Read the model definition and answer for the solid it produces. Units are mm, in the model's axes. A direction names the side the tool comes from. Coordinates: 2 decimals unless noted, no trailing zeros. Write each loop counter-clockwise with the first axis right and the second up, starting at its lowest first coordinate (ties: lowest second). Pieces come first, ordered by that corner, then holes.
from build123d import *

# Parameters (mm, degrees)
BASE_PLATE_PROFILE_R      = 7.492267371
BASE_PLATE_20MM_DEPTH     = 20
HINGE_KNUCKLE_PROFILE_R   = 10.5
HINGE_KNUCKLE_145MM_DEPTH = 72.5


with BuildPart() as part:
    # Base Plate Profile → Base Plate 20mm (new body)
    with BuildSketch(Plane.XY):
        with BuildLine():
            Line((-72.5, 28.064546487), (72.5, 28.064546487))
            Line((72.5, 28.064546487), (72.5, -16.935453513))
            ThreePointArc((72.5, -16.935453513), (69.894587599, -26.538447706), (62.792895003, -33.507782934))
            Line((62.792895003, -33.507782934), (9.292895003, -63.507782934))
            ThreePointArc((9.292895003, -63.507782934), (0, -65.935453513), (-9.292895003, -63.507782934))
            Line((-9.292895003, -63.507782934), (-62.792895003, -33.507782934))
            ThreePointArc((-62.792895003, -33.507782934), (-69.894587599, -26.538447706), (-72.5, -16.935453513))
            Line((-72.5, -16.935453513), (-72.5, 28.064546487))
        make_face()
        with Locations((0, -46.935453513)):
            Circle(BASE_PLATE_PROFILE_R, mode=Mode.SUBTRACT)
        with Locations((53.5, -16.935453513)):
            Circle(BASE_PLATE_PROFILE_R, mode=Mode.SUBTRACT)
        with Locations((-53.5, -16.935453513)):
            Circle(BASE_PLATE_PROFILE_R, mode=Mode.SUBTRACT)
    extrude(amount=BASE_PLATE_20MM_DEPTH)

    # Hinge Knuckle Profile → Hinge Knuckle 145mm (add, symmetric)
    with BuildSketch(Plane(origin=(0, 0, 0), x_dir=(0, 0, -1), z_dir=(1, 0, 0))):
        with BuildLine():
            Line((29, 61.064546487), (29, 28.064546487))
            Line((29, 28.064546487), (-13, 28.064546487))
            Line((-13, 28.064546487), (-13, 61.064546487))
            ThreePointArc((-13, 61.064546487), (8, 82.064546487), (29, 61.064546487))
        make_face()
        with Locations((8, 61.064546487)):
            Circle(HINGE_KNUCKLE_PROFILE_R, mode=Mode.SUBTRACT)
    extrude(amount=HINGE_KNUCKLE_145MM_DEPTH, both=True)


solid = part.part
Item 1: Determine the mould class of faces 1 (the cylindrical face through (-0.975, -39.507, 9.86)), 2 (the flat face through (72.5, 33, 1)), 3 (the cylindrical face through (-1.015, 54.675, 0.332)) for opening direction X: +X half, -X half, draft (parallel to the pull), parting line (faces both ways), or undercut.
Item 2: The part is cut by section A-A (x = 0). Give the vertices of the cut face in (y, z).
Item 3: The part is cut by section B-B (z = -8). Give the vertices of the cut face in (x, y), and give its area (4 significant figures).
Item 4: Given pin 1 (19.5 mm diameter, centred on x = 0, y = -46.94, fed in from -Z); pin 2 (4 mm diameter, centred on x = 22, z = -16, fed in from +Y); pin 3 (12 mm diameter, centred on x = 35.5, z = -6, fed in from +Y); pin 4 (24 mm diameter, centred on x = -53.5, y = -16.94, fed in from +Z), each flat-ended and moving along its own axis, determine where each tip first touches the part or whether it passes through.
Item 5: Find the intervals of material crossed by probe 1 along Y at (x, z) = (0, -8); probe 2 along Z at (x, y) = (26.5, 17.5); probe 3 along Z at (x, y) = (32.5, 48), in increasing order.
Item 6: The part is cut by section C-C (z = 9). Give the vertices of the cut face in (x, y).
Item 7: The part is cut by section D-D (x = 30.5). Give the vertices of the cut face in (y, z), and give its area (3 significant figures).
Item 8: For faces 4 (the cylindrical face through (69.965, -26.417, 9.86)), 5 (the flat face through (1, 28.065, -15)), 6 (the flat face through (1, 44, 13)), determine the directions among +Z, -Z, +X, -X, +Y, -Y from which every point of the face is accessible in a straight line to the end or side of a thin tool.
Answer:
1. face 1: undercut
1. face 2: +X half
1. face 3: draft
2. outline: (-65.94, 0) - (-54.43, 0) - (-54.43, 20) - (-65.94, 20) - close; (-39.44, 0) - (28.06, 0) - (28.06, -29) - (61.06, -29) arc R21 ccw to (61.06, 13) - (28.06, 13) - (28.06, 20) - (-39.44, 20) - close; hole circle Ø21 at (61.06, -8)
3. outline: (-72.5, 28.06) - (72.5, 28.06) - (72.5, 50.56) - (-72.5, 50.56) - close; (-72.5, 71.56) - (72.5, 71.56) - (72.5, 82.06) - (-72.5, 82.06) - close
3. area: 4,785 mm2
4. pin 1: stops at z = 0
4. pin 2: stops at y = 81.19
4. pin 3: stops at y = 82.06
4. pin 4: stops at z = 20
5. probe 1: y = 28.06 to 50.56, 71.56 to 82.06
5. probe 2: z = 0 to 20
5. probe 3: z = -29 to 13
6. outline: (-72.5, -16.94) arc R19 ccw to (-62.79, -33.51) - (-9.29, -63.51) arc R19 ccw to (9.29, -63.51) - (62.79, -33.51) arc R19 ccw to (72.5, -16.94) - (72.5, 73.39) - (-72.5, 73.39) - close; hole circle Ø14.98 at (-53.5, -16.94); hole circle Ø14.98 at (0, -46.94); hole circle Ø14.98 at (53.5, -16.94)
7. outline: (-51.62, 0) - (28.06, 0) - (28.06, -29) - (61.06, -29) arc R21 ccw to (61.06, 13) - (28.06, 13) - (28.06, 20) - (-51.62, 20) - close; hole circle Ø21 at (61.06, -8)
7. area: 3,330 mm2
8. face 4: +Z, -Z, +X, -Y
8. face 5: -Z, +X, -X, -Y
8. face 6: +Z, +X, -X, +Y
